from build123d import *

# Parameters (mm, degrees)
SKETCH1_R           = 25
BOSS_EXTRUDE1_DEPTH = 9
SKETCH2_R           = 18
CUT_EXTRUDE1_DEPTH  = 4
SKETCH3_R           = 5
CUT_EXTRUDE2_DEPTH  = 36.707142143
SKETCH4_R           = 4
CUT_EXTRUDE3_DEPTH  = 36.707142143
SKETCH5_R           = 6
SKETCH5_R_2         = 4
BOSS_EXTRUDE2_DEPTH = 1


with BuildPart() as part:
    # Sketch1 → Boss-Extrude1 (new body)
    with BuildSketch(Plane.XY):
        Circle(SKETCH1_R)
    extrude(amount=BOSS_EXTRUDE1_DEPTH)

    # Sketch2 → Cut-Extrude1 (cut)
    with BuildSketch(Plane.XY.offset(9)):
        Circle(SKETCH2_R)
    extrude(amount=-CUT_EXTRUDE1_DEPTH, mode=Mode.SUBTRACT)

    # Sketch3 → Cut-Extrude2 (cut, through all)
    with BuildSketch(Plane.XY.offset(5)):
        with Locations((0, 12)):
            Circle(SKETCH3_R)
        with Locations((12, 0)):
            Circle(SKETCH3_R)
        with Locations((0, -12)):
            Circle(SKETCH3_R)
        with Locations((-12, 0)):
            Circle(SKETCH3_R)
    extrude(amount=-CUT_EXTRUDE2_DEPTH, mode=Mode.SUBTRACT)

    # Sketch4 → Cut-Extrude3 (cut, through all)
    with BuildSketch(Plane.XY.offset(5)):
        Circle(SKETCH4_R)
    extrude(amount=-CUT_EXTRUDE3_DEPTH, mode=Mode.SUBTRACT)

    # Sketch5 → Boss-Extrude2 (add)
    with BuildSketch(Plane(origin=(0, 0, 0), x_dir=(-1, 0, 0), z_dir=(0, 0, -1))):
        with Locations(Location((0, 0, 0), (0, 0, 180))):
            Circle(SKETCH5_R)
        with Locations(Location((0, 0, 0), (0, 0, 180))):
            Circle(SKETCH5_R_2, mode=Mode.SUBTRACT)
    extrude(amount=BOSS_EXTRUDE2_DEPTH)


solid = part.part
The listing builds one solid part. Answer for the finished solid, in the listing's coordinates (mm). A direction names the side the tool comes from. Give positions to 0.01 mm unless a question says otherwise; leave off trailing zeros. Loops run counter-clockwise (first coordinate to the right, second up) from the corner with the lowest first, then second, coordinate; pieces in that order, holes last. Notation, with made-up numbers: (-3.5, -27.5) - (33.5, -27.5) arc R13 cw to (33.5, -2.5) - close; hole circle Ø7 at (51.5, 73). An arc over 180 degrees is marked (long way). Write each question's results on one line, items separated by ' | '.
1. Find section C-C, the plane z = 4.25. Write down the section's boundary in (x, y).
Resolved:
outline: circle Ø50 at (0, 0); hole circle Ø10 at (-12, 0); hole circle Ø10 at (0, -12); hole circle Ø10 at (0, 12); hole circle Ø8 at (0, 0); hole circle Ø10 at (12, 0)
2. Find section B-B, the plane x = 13.5. Write down the section's boundary in (y, z), then the cut area to 3 significant figures.
Resolved:
outline: (-21.04, 0) - (-4.77, 0) - (-4.77, 5) - (-11.91, 5) - (-11.91, 9) - (-21.04, 9) - close; (4.77, 0) - (21.04, 0) - (21.04, 9) - (11.91, 9) - (11.91, 5) - (4.77, 5) - close | area: 236 mm^2
3. Find section A-A, the plane y = 0. Write down the section's boundary in (x, z), then the cut area to 3 significant figures.
Resolved:
outline: (-25, 0) - (-17, 0) - (-17, 5) - (-18, 5) - (-18, 9) - (-25, 9) - close; (-7, 0) - (-6, 0) - (-6, -1) - (-4, -1) - (-4, 5) - (-7, 5) - close; (4, -1) - (6, -1) - (6, 0) - (7, 0) - (7, 5) - (4, 5) - close; (17, 0) - (25, 0) - (25, 9) - (18, 9) - (18, 5) - (17, 5) - close | area: 170 mm^2
4. For a pull along X with two mould halves and no side action, classify faces 1 (the face through (-4.3, 0.3, 5)), 2 (the face through (11, -16, 9)), 3 (the face through (23.846, 7.509, 4.437)) as +X half, -X half, draft (parallel to the pull), parting line (faces both ways), or undercut.
Resolved:
face 1: undercut | face 2: draft | face 3: parting line
5. Flat-ended cylindrical pins translate along their axes: P1, Ø7, axis at x = 0, y = 0, coming from the +Z side (3 decimals); P2, Ø2, axis at x = -20, z = 7, coming from the -Y side; P3, Ø1, axis at x = -9, z = 3, coming from the -Y side; P4, Ø6, axis at y = 17, z = 8, coming from the -X side. Find the tip coordinate at first contact, or state that the pin passes through.
Resolved:
P1: passes through | P2: stops at y = -16.25 | P3: stops at y = -23.51 | P4: stops at x = -20.71
6. Which of the six approach directions +Z, -Z, +X, -X, +Y, -Y give full straight-line access (tool end or side, diameter ignored) to faces 4 (the face through (5.723, -1.802, -0.493)), 5 (the face through (-2.343, 17.847, 7.028)), 6 (the face through (3.92, -1.42, -1))?
Resolved:
face 4: -Z | face 5: +Z | face 6: -Z, +X, -X, +Y, -Y
7. Consider probe 1 along Y at (x, z) = (0, 2.35); probe 2 along Y at (x, z) = (0, 6.6); probe 3 along Z at (x, y) = (4, 2). Determine where each line is inside the solid, lowest interval first. Write a range as from..to.
Resolved:
probe 1: y = -25..-17, -7..-4, 4..7, 17..25 | probe 2: y = -25..-18, 18..25 | probe 3: z = -1..5
8. Find section D-D, the plane x = 0.5. Write down the section's boundary in (y, z) (3 decimals).
Resolved:
outline: (-24.995, 0) - (-16.975, 0) - (-16.975, 5) - (-17.993, 5) - (-17.993, 9) - (-24.995, 9) - close; (-7.025, 0) - (-5.979, 0) - (-5.979, -1) - (-3.969, -1) - (-3.969, 5) - (-7.025, 5) - close; (3.969, -1) - (5.979, -1) - (5.979, 0) - (7.025, 0) - (7.025, 5) - (3.969, 5) - close; (16.975, 0) - (24.995, 0) - (24.995, 9) - (17.993, 9) - (17.993, 5) - (16.975, 5) - close
